CAD build for the part. Positions are in the model's coordinates, mm. Give positions to 0.01 mm unless a question says otherwise; leave off trailing zeros. Loops run counter-clockwise (first coordinate to the right, second up) from the corner with the lowest first, then second, coordinate; pieces in that order, holes last. Notation, with made-up numbers: (-25, -8) -> (-13, -8) arc R20 cw to (-13, 8) -> close; hole circle Ø8 at (-18, 71.5). An arc over 180 degrees is marked (long way). Write each question's results on one line, items separated by ' | '. Start each with the question number.
```python
from build123d import *

# Parameters (mm, degrees)
LINK_PROFILE_R       = 5
LINK_PLATE_5MM_DEPTH = 5


with BuildPart() as part:
    # Link Profile → Link Plate 5mm (new body)
    with BuildSketch(Plane(origin=(0, 0, 0), x_dir=(1, 0, 0), z_dir=(0, 1, 0))):
        with BuildLine():
            Line((-15, 10), (15, 10))
            ThreePointArc((15, 10), (25, 0), (15, -10))
            Line((15, -10), (-15, -10))
            ThreePointArc((-15, -10), (-25, 0), (-15, 10))
        make_face()
        with Locations(Location((-15, 0, 0), (0, 0, 270))):
            Circle(LINK_PROFILE_R, mode=Mode.SUBTRACT)
        with Locations(Location((15, 0, 0), (0, 0, 270))):
            Circle(LINK_PROFILE_R, mode=Mode.SUBTRACT)
    extrude(amount=LINK_PLATE_5MM_DEPTH)


solid = part.part
```
Q1. Saw through at A-A, the plane z = 0. List the corners of the cut face in (x, y), then the cut area to 3 significant figures.
Q2. Wall check: L1, parallel to X at y = 3.4, z = 0; L2, parallel to X at y = 2.85, z = -3.5; L3, parallel to Z at x = 18.5, y = 4.4. Give the ranges that are in metal, low to high.
Q3. Mould opens along Z. For faces 1 (the face through (0, 5, 0)), 2 (the face through (0, 2, -10)), 3 (the face through (10.12, 2.46, -1.08)), 4 (the face through (-19.88, 2.46, -1.08)) say: pulls with the +Z half, pulls with the -Z half, needs draft (parallel to the pull), parting line crosses it, or undercut.
Q4. Saw through at B-B, the plane x = 19. List the corners of the cut face in (y, z).
Q5. Saw through at C-C, the plane y = 4.15. List the corners of the cut face in (x, z).
Q6. Saw through at D-D, the plane z = 2. List the corners of the cut face in (x, y).
Answer block:
1) outline: (-25, 0) -> (-20, 0) -> (-20, 5) -> (-25, 5) -> close; (-10, 0) -> (10, 0) -> (10, 5) -> (-10, 5) -> close; (20, 0) -> (25, 0) -> (25, 5) -> (20, 5) -> close | area: 150 mm2
2) L1: x = -25 to -20, -10 to 10, 20 to 25 | L2: x = -24.37 to -18.57, -11.43 to 11.43, 18.57 to 24.37 | L3: z = -9.37 to -3.57, 3.57 to 9.37
3) face 1: needs draft | face 2: pulls with the -Z half | face 3: undercut | face 4: undercut
4) outline: (0, -9.17) -> (5, -9.17) -> (5, -3) -> (0, -3) -> close; (0, 3) -> (5, 3) -> (5, 9.17) -> (0, 9.17) -> close
5) outline: (-15, -10) -> (15, -10) arc R10 ccw to (15, 10) -> (-15, 10) arc R10 ccw to start; hole circle Ø10 at (-15, 0); hole circle Ø10 at (15, 0)
6) outline: (-24.8, 0) -> (-19.58, 0) -> (-19.58, 5) -> (-24.8, 5) -> close; (-10.42, 0) -> (10.42, 0) -> (10.42, 5) -> (-10.42, 5) -> close; (19.58, 0) -> (24.8, 0) -> (24.8, 5) -> (19.58, 5) -> close
